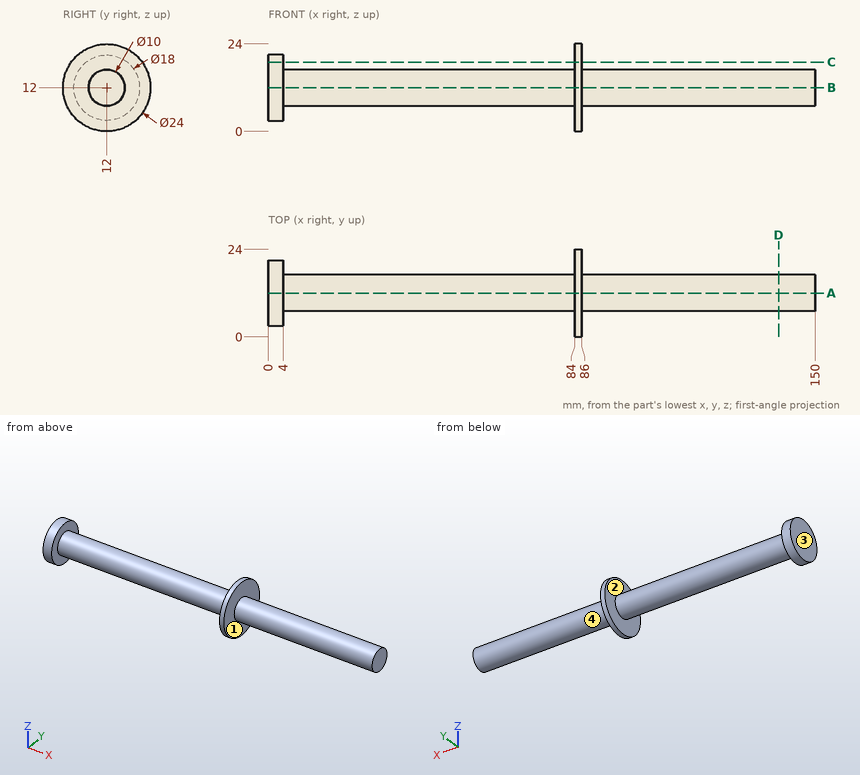
The figure shows three views and two pictorial views of one solid part (mm, origin at its lowest corner). Answer the questions. Give positions to 0.01 mm unless a question says otherwise; leave off trailing zeros. Order: outer loops, then holes, each group sorted by start corner. A loop starts at its lowest first (then second) coordinate and runs counter-clockwise, first axis right, second up. Notation, with made-up numbers: (36.5, 8.5) -> (59.5, 8.5) arc R16 ccw to (59.5, 20.5) -> close; hole circle Ø4 at (85.25, 29). An arc over 180 degrees is marked (long way). Answer as CSV lines item,"result". Start each with the question number.
(1) Section D-D, the plane x = 140 is taken. Write down the section's boundary in (y, z).
(2) Consider line 1 along X through (y, z) = (5.75, 15); line 2 along X through (y, z) = (2.25, 18); line 3 along Z through (x, y) = (86.5, 11.75). Determine where each line is inside the solid, lowest interval first.
(3) Section C-C, the plane z = 19 is taken. Write down the section's boundary in (x, y), plus the area to 3 significant figures.
(4) For a pull along X with two mould halves and no side action, classify the marked faces 1, 2, 3 and 4 as released by +X, released by -X, zero draft, split by the parting line, or undercut.
(5) Section A-A, the plane y = 12 is taken. Write down the section's boundary in (x, z).
(6) Each of these flat-tipped pins is pushed along its axis until it touches: pin 1 Ø1.5 at (x, y) = (117, 14) entering from -Z; pin 2 Ø8 at (x, z) = (18.5, 6.5) entering from +Y; pin 3 Ø1.5 at (x, z) = (111, 16.5) entering from +Y. Where does it stop, or does it pass through?
Entries:
1,outline,"circle Ø10 at (12, 12)"
2,line 1,"0 to 4, 84 to 86"
2,line 2,"84 to 86"
2,line 3,"7.01 to 16.99"
3,outline,"(0, 6.34) -> (4, 6.34) -> (4, 17.66) -> (0, 17.66) -> close; (84, 2.25) -> (86, 2.25) -> (86, 21.75) -> (84, 21.75) -> close"
3,area,"84.2 mm²"
4,face 1,"released by +X"
4,face 2,"undercut"
4,face 3,"released by -X"
4,face 4,"zero draft"
5,outline,"(0, 3) -> (4, 3) -> (4, 7) -> (84, 7) -> (84, 0) -> (86, 0) -> (86, 7) -> (150, 7) -> (150, 17) -> (86, 17) -> (86, 24) -> (84, 24) -> (84, 17) -> (4, 17) -> (4, 21) -> (0, 21) -> close"
6,pin 1,"z = 7.16"
6,pin 2,"y = 16.77"
6,pin 3,"y = 15.31"
